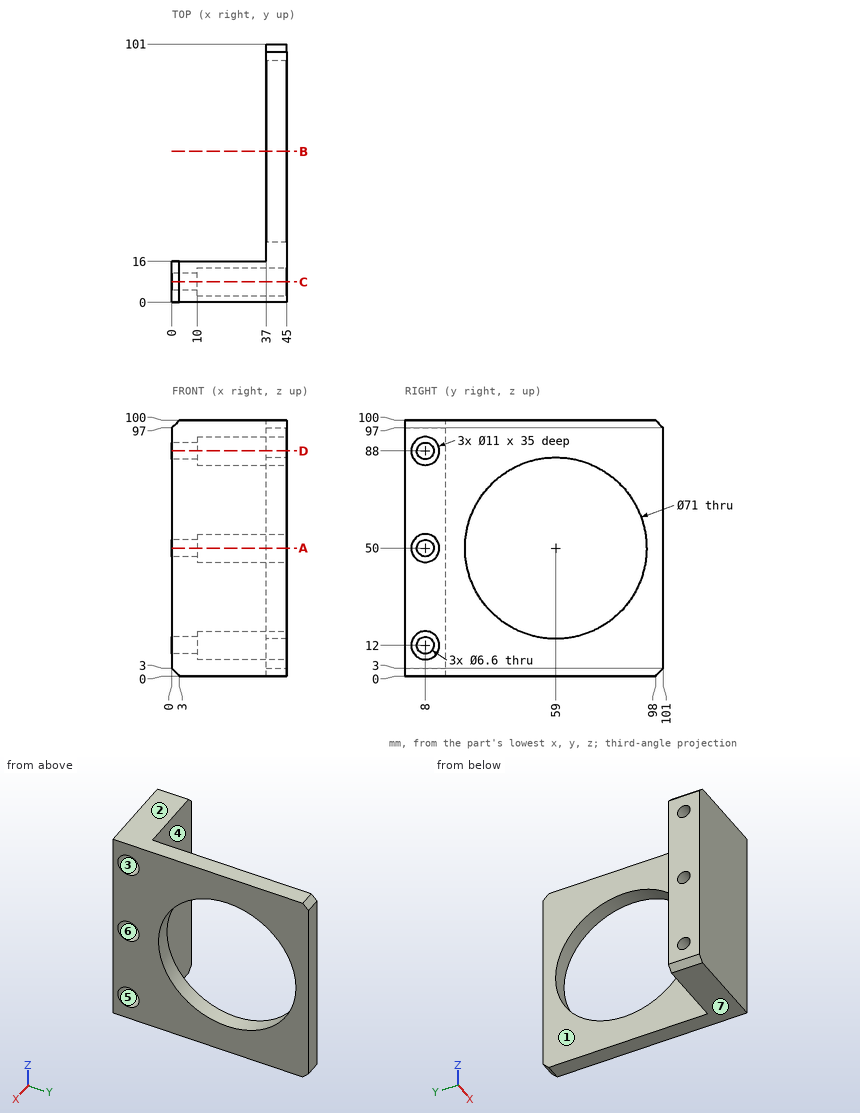
Source: three-view drawing plus pictorial views. Frame: mm from the lowest corner of the part. A direction names the side the tool comes from. Give positions to 0.01 mm unless a question says otherwise; leave off trailing zeros. Loops run counter-clockwise (first coordinate to the right, second up) from the corner with the lowest first, then second, coordinate; pieces in that order, holes last.
1) Line query: L1, parallel to Z at x = 3.5, y = 8; L2, parallel to Y at x = 5.25, z = 12; L3, parallel to X at y = 28.5, z = 90.5. Output: solid intervals per line, ascending.
A:
L1: z = 0 to 8.7, 15.3 to 46.7, 53.3 to 84.7, 91.3 to 100
L2: y = 0 to 4.7, 11.3 to 16
L3: x = 37 to 45
2) Section query C-C on y = 8. Count the separate pieces of the cut face and the enclosed holes in it, and give its area (3 significant figures).
A:
separate pieces: 4
enclosed holes: 0
area: 3,140 mm2
3) Section query D-D on z = 88. Return the cut outline in (x, y).
A:
outline: (0, 0) - (45, 0) - (45, 2.5) - (10, 2.5) - (10, 4.7) - (0, 4.7) - close; (0, 11.3) - (10, 11.3) - (10, 13.5) - (45, 13.5) - (45, 101) - (37, 101) - (37, 16) - (0, 16) - close
4) Section query B-B on y = 59. Return the cut outline in (x, z).
A:
outline: (37, 0) - (45, 0) - (45, 14.5) - (37, 14.5) - close; (37, 85.5) - (45, 85.5) - (45, 100) - (37, 100) - close
5) Mould query, pull axis Z, two halves, no side actions, for the marked faces 4, 5, 6 and 7. Classes: released by +Z, released by -Z, zero draft, split by the parting line, or undercut.
A:
face 4: zero draft
face 5: undercut
face 6: undercut
face 7: released by -Z
6) Section query A-A on z = 50. Return the cut outline in (x, y).
A:
outline: (0, 0) - (45, 0) - (45, 2.5) - (10, 2.5) - (10, 4.7) - (0, 4.7) - close; (0, 11.3) - (10, 11.3) - (10, 13.5) - (45, 13.5) - (45, 23.5) - (37, 23.5) - (37, 16) - (0, 16) - close; (37, 94.5) - (45, 94.5) - (45, 101) - (37, 101) - close
7) Contact query for flat-ended pins moving along their axis: pin 1 (10 mm diameter, centred on y = 8, z = 88, fed in from +X); pin 2 (6 mm diameter, centred on y = 26.5, z = 79, fed in from -X). Output: stop coordinate, or through.
A:
pin 1: stops at x = 10
pin 2: stops at x = 37
8) Reachability of the marked faces 1, 2 and 3 from +Z, -Z, +X, -X, +Y, -Y: full face, straight path, thin tool, end or side. Return the list, or none.
A:
face 1: +Z, -Z, -X, +Y
face 2: +Z, +X, -X, +Y, -Y
face 3: +X
